```python
from build123d import *

# Parameters (mm, degrees)
SKETCH_1_W          = 20
SKETCH_1_H          = 10
EXTRUDE_1_DEPTH     = 8
SKETCH_2_R          = 1
CUT_EXTRUDE_1_DEPTH = 8
CHAMFER_1_SIZE      = 2
SKETCH_3_R          = 4
EXTRUDE_2_DEPTH     = 1
SKETCH_4_R          = 2.5
EXTRUDE_3_DEPTH     = 5
FILLET_1_R          = 2.5


with BuildPart() as part:
    # 草图1 → 凸台-拉伸1 (new body)
    with BuildSketch(Plane.XY):
        with Locations((10, 5)):
            Rectangle(SKETCH_1_W, SKETCH_1_H)
    extrude(amount=EXTRUDE_1_DEPTH)

    # 草图2 → 切除-拉伸1 (cut)
    with BuildSketch(Plane.XY.offset(8)):
        with Locations((5, 5)):
            Circle(SKETCH_2_R)
    extrude(amount=-CUT_EXTRUDE_1_DEPTH, mode=Mode.SUBTRACT)

    # 倒角1
    chamfer_1_edges = [part.edges().sort_by_distance(p)[0] for p in [
        (4, 5, 8),
    ]]
    chamfer(chamfer_1_edges, length=CHAMFER_1_SIZE)

    # 草图3 → 凸台-拉伸2 (add)
    with BuildSketch(Plane.XY.offset(8)):
        with Locations(Location((15, 5, 0), (0, 0, 180))):
            Circle(SKETCH_3_R)
    extrude(amount=EXTRUDE_2_DEPTH)

    # 草图4 → 凸台-拉伸3 (add)
    with BuildSketch(Plane.XY.offset(9)):
        with Locations((15, 5)):
            Circle(SKETCH_4_R)
    extrude(amount=EXTRUDE_3_DEPTH)

    # 圆角1
    fillet_1_edges = [part.edges().sort_by_distance(p)[0] for p in [
        (12.5, 5, 14),
    ]]
    fillet(fillet_1_edges, radius=FILLET_1_R)


solid = part.part
```
Read the model definition and answer for the solid it produces. Units are mm, in the model's axes. A direction names the side the tool comes from. Coordinates: 2 decimals unless noted, no trailing zeros. Write each loop counter-clockwise with the first axis right and the second up, starting at its lowest first coordinate (ties: lowest second). Pieces come first, ordered by that corner, then holes. Notation, with made-up numbers: (-0.75, 76.25) -> (47.25, 76.25) arc R16 ccw to (47.25, 80.25) -> close; hole circle Ø3 at (73.25, 36.25). An arc over 180 degrees is marked (long way). Return JSON: item names as keys, results as strings.
1. A cutting plane is placed at A-A (x = 5). Determine the outline of the cut face in (y, z).
Found:
{"outline": "(0, 0) -> (4, 0) -> (4, 6) -> (2, 8) -> (0, 8) -> close; (6, 0) -> (10, 0) -> (10, 8) -> (8, 8) -> (6, 6) -> close"}
2. A cutting plane is placed at C-C (x = 15). Determine the outline of the cut face in (y, z).
Found:
{"outline": "(0, 0) -> (10, 0) -> (10, 8) -> (9, 8) -> (9, 9) -> (7.5, 9) -> (7.5, 11.5) arc R2.5 ccw to (2.5, 11.5) -> (2.5, 9) -> (1, 9) -> (1, 8) -> (0, 8) -> close"}
3. A tool of negligible diameter and unlimited length cuts with its end or side. For faces 1 (the face through (18.996, 4.824, 8.493)), 2 (the face through (10, 5, 0)), from which of +Z, -Z, +X, -X, +Y, -Y can it reach the whole face along a straight path? Write none if from no direction.
Found:
{"face 1": "+Z", "face 2": "-Z, +X, -X, +Y, -Y"}
4. A cutting plane is placed at D-D (z = 9.75). Determine the outline of the cut face in (x, y).
Found:
{"outline": "circle Ø5 at (15, 5)"}
5. A cutting plane is placed at B-B (y = 5). Determine the outline of the cut face in (x, z).
Found:
{"outline": "(0, 0) -> (4, 0) -> (4, 6) -> (2, 8) -> (0, 8) -> close; (6, 0) -> (20, 0) -> (20, 8) -> (19, 8) -> (19, 9) -> (17.5, 9) -> (17.5, 11.5) arc R2.5 ccw to (12.5, 11.5) -> (12.5, 9) -> (11, 9) -> (11, 8) -> (8, 8) -> (6, 6) -> close"}
6. Each of these flat-tipped pins is pushed along its axis until it touches: P1, Ø3, axis at y = 5, z = 11.5, coming from the -X side; P2, Ø1.2, axis at x = 5, y = 5, coming from the -Z side. Where does it stop, or does it pass through?
Found:
{"P1": "x = 12.5", "P2": "through"}
7. Find the intervals of material crossed by line 1 along Y through (x, z) = (5, 2.3); line 2 along Y through (x, z) = (5, 7.5); line 3 along Z through (x, y) = (8, 8.25), in increasing order. Write a range as from..to.
Found:
{"line 1": "0..4, 6..10", "line 2": "0..2.5, 7.5..10", "line 3": "0..8"}
8. Determine the mould class of faces 3 (the face through (5, 6, 3)), 4 (the face through (20, 5, 4)), 5 (the face through (12.5, 5.1, 10.2)), 6 (the face through (10, 0, 4)) for opening direction X: pulls with the +X half, pulls with the -X half, needs draft (parallel to the pull), parting line crosses it, or undercut.
Found:
{"face 3": "undercut", "face 4": "pulls with the +X half", "face 5": "parting line crosses it", "face 6": "needs draft"}
